The listing builds one solid part. Answer for the finished solid, in the listing's coordinates (mm). A direction names the side the tool comes from. Round coordinates to 2 decimals unless told otherwise and drop trailing zeros. Order: outer loops, then holes, each group sorted by start corner. A loop starts at its lowest first (then second) coordinate and runs counter-clockwise, first axis right, second up. Notation, with made-up numbers: M 55.25,40.5 L 91.25,40.5 A35 ccw 91.25,79.5 Z; hole C -23.5,42 d6. An arc over 180 degrees is marked long. Put each result on its own line as item: value. Start each with the question number.
1. Each of these flat-tipped pins is pushed along its axis until it touches: pin 1 Ø5 at (y, z) = (86.5, -20) entering from -X; pin 2 Ø4 at (x, y) = (55, 40) entering from -Z; pin 3 Ø9 at (x, z) = (8, -9) entering from +Y; pin 4 Ø8 at (x, y) = (49, 56.5) entering from -Z. Where does it stop, or does it pass through?
2. The part is cut by section B-B (x = 101.25). Give the vertices of the cut face in (y, z).
3. The part is cut by section A-A (z = -14.5). Count the separate pieces of the cut face and the enclosed holes in it, then the cut area to 3 significant figures.
4. Which of the six approach directions +Z, -Z, +X, -X, +Y, -Y give full straight-line access (tool end or side, diameter ignored) to faces 5 (the face through (56.94, 99.2, -17.71)), 6 (the face through (93.6, 70, -12.2)), 7 (the face through (93.93, 42.89, -13.63))?
5. Consider line 1 (Y direction, x = 55, z = -15.25); line 2 (X direction, y = 20, z = -18); line 3 (X direction, y = 24, z = -11.5). Determine where each line is inside the solid, lowest interval first.
6. The mould has two halves that part along Y. Classify faces 1 (the face through (69, 53, -5)), 2 (the face through (17.5, 80, -12)), 3 (the face through (96, 15, -12)), 4 (the face through (84.832, 69.676, -10.557)): +Y half, -Y half, draft (parallel to the pull), parting line (faces both ways), or undercut.
7. The part is cut by section D-D (x = 20.5). Give the vertices of the cut face in (y, z).
from build123d import *

# Parameters (mm, degrees)
SKETCH_1_W                = 110
SKETCH_1_H                = 24
EXTRUDE_1_DEPTH           = 110
SKETCH_2_R                = 21
CUT_EXTRUDE_1_DEPTH       = 5
SKETCH_3_R                = 23.5
CUT_EXTRUDE_2_DEPTH       = 19
SKETCH_5_W                = 17.5
SKETCH_5_H                = 40
CUT_EXTRUDE_3_DEPTH       = 158.40393896
CHAMFER_1_SIZE            = 20
HOLE_WIZARD_M5_1_D        = 4.2
HOLE_WIZARD_M5_1_DEPTH    = 12.4
HOLE_WIZARD_M5_1_TIP      = 1.2618073
HOLE_WIZARD_1_D           = 9
HOLE_WIZARD_1_CBORE_D     = 15
HOLE_WIZARD_1_CBORE_DEPTH = 55
FILLET_2_R                = 0.5
CHAMFER_2_SIZE            = 0.5


with BuildPart() as part:
    # 草图1 → 拉伸1 (new body)
    with BuildSketch(Plane(origin=(0, 0, 0), x_dir=(1, 0, 0), z_dir=(0, 1, 0))):
        with Locations((55, 12)):
            Rectangle(SKETCH_1_W, SKETCH_1_H)
    extrude(amount=EXTRUDE_1_DEPTH)

    # 草图2 → 切除-拉伸1 (cut)
    with BuildSketch(Plane.XY):
        with Locations((55, 70)):
            Circle(SKETCH_2_R)
    extrude(amount=-CUT_EXTRUDE_1_DEPTH, mode=Mode.SUBTRACT)

    # 草图3 → 切除-拉伸2 (cut)
    with BuildSketch(Plane.XY.offset(-5)):
        with Locations((55, 70)):
            Circle(SKETCH_3_R)
    extrude(amount=-CUT_EXTRUDE_2_DEPTH, mode=Mode.SUBTRACT)

    # 草图5 → 切除-拉伸3 (cut, through all)
    with BuildSketch(Plane(origin=(0, 0, -24), x_dir=(-1, 0, 0), z_dir=(0, 0, -1))):
        with Locations((-101.25, 90)):
            Rectangle(SKETCH_5_W, SKETCH_5_H)
        with Locations((-8.75, 90)):
            Rectangle(SKETCH_5_W, SKETCH_5_H)
    extrude(amount=-CUT_EXTRUDE_3_DEPTH, mode=Mode.SUBTRACT)

    # 倒角1
    chamfer_1_edges = [part.edges().sort_by_distance(p)[0] for p in [
        (92.5, 110, -12),
        (17.5, 110, -12),
    ]]
    chamfer(chamfer_1_edges, length=CHAMFER_1_SIZE)

    # M5 螺纹孔1
    with Locations(Plane(origin=(55, 100, -24), x_dir=(-1, 0, 0), z_dir=(0, 0, -1))):
        with Locations((0, 0), (-30, -30), (0, -60), (30, -30)):
            Hole(HOLE_WIZARD_M5_1_D / 2, depth=HOLE_WIZARD_M5_1_DEPTH)
            with Locations((0, 0, -(HOLE_WIZARD_M5_1_DEPTH + HOLE_WIZARD_M5_1_TIP / 2))):  # 118° drill point
                Cone(0, HOLE_WIZARD_M5_1_D / 2, HOLE_WIZARD_M5_1_TIP, mode=Mode.SUBTRACT)

    # 打孔尺寸根据内六角圆柱头螺钉的类型1 (through all)
    with Locations(Plane(origin=(8.75, 70, -12), x_dir=(0, 0, 1), z_dir=(0, 1, 0))):
        with Locations((0, 0), (0, 92.5)):
            CounterBoreHole(HOLE_WIZARD_1_D / 2, HOLE_WIZARD_1_CBORE_D / 2, HOLE_WIZARD_1_CBORE_DEPTH)

    # 圆角2
    fillet_2_edges = [part.edges().sort_by_distance(p)[0] for p in [
        (34, 70, 0),
        (31.5, 70, -5),
        (34, 70, -5),
    ]]
    fillet(fillet_2_edges, radius=FILLET_2_R)

    # 倒角2
    chamfer_2_edges = [part.edges().sort_by_distance(p)[0] for p in [
        (31.5, 70, -24),
    ]]
    chamfer(chamfer_2_edges, length=CHAMFER_2_SIZE)


solid = part.part
Resolved:
1. pin 1: x = 17.5
1. pin 2: z = -11.54
1. pin 3: y = 70
1. pin 4: through
2. outline: M 0,-24 L 70,-24 L 70,-19.5 L 15,-19.5 L 15,-16.5 L 0,-16.5 Z; M 0,-7.5 L 15,-7.5 L 15,-4.5 L 70,-4.5 L 70,0 L 0,0 Z
3. separate pieces: 3
3. enclosed holes: 5
3. area: 6,730 mm2
4. face 5: -Z
4. face 6: +Z, -Z, +X, +Y
4. face 7: +Y
5. line 1: 0 to 37.9, 42.1 to 46.5, 93.5 to 97.9, 102.1 to 110
5. line 2: 0 to 4.25, 13.25 to 96.75, 105.75 to 110
5. line 3: 0 to 1.27, 16.23 to 93.77, 108.73 to 110
6. face 1: undercut
6. face 2: draft
6. face 3: +Y half
6. face 4: undercut
7. outline: M 0,-24 L 93,-24 L 93,0 L 0,0 Z
